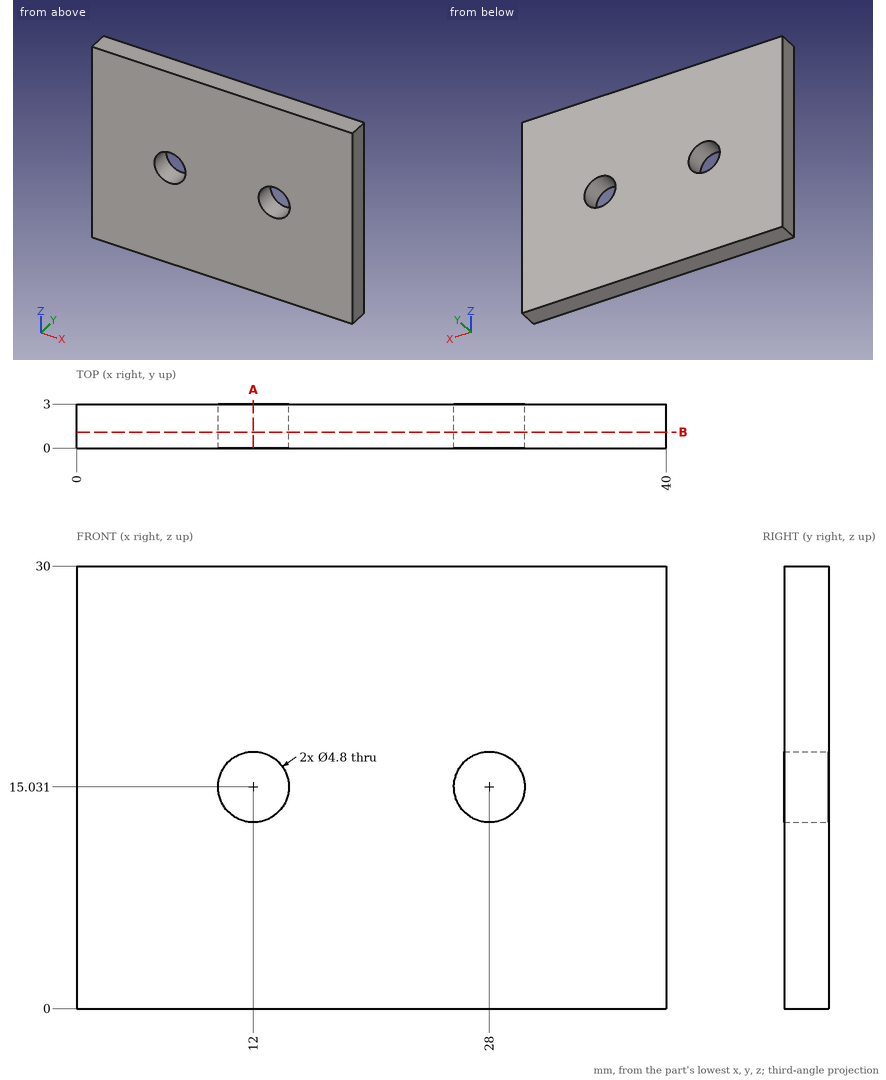
Geometry: see drawing. Coordinates: mm, zero at the bounding-box minimum. Coordinates: 2 decimals unless noted, no trailing zeros. Write each loop counter-clockwise with the first axis right and the second up, starting at its lowest first coordinate (ties: lowest second). Pieces come first, ordered by that corner, then holes. Notation, with made-up numbers: (26.25, 24.25) - (49.25, 24.25) arc R30 ccw to (49.25, 56.25) - close; hole circle Ø8 at (40, 67). An arc over 180 degrees is marked (long way). Put each result on its own line as item: value. Start each with the question number.
1) Ray query, L1, parallel to X at y = 1.65, z = 13.75; L2, parallel to Z at x = 27, y = 1.75; L3, parallel to Z at x = 29.5, y = 0.7. Return the intervals inside material, ascending.
2) Cut plane B-B (y = 1.1). Return the cut outline in (x, z), plus the area to 3 significant figures.
3) Cut plane A-A (x = 12). Return the cut outline in (y, z).
Resolved:
1. L1: x = 0 to 9.97, 14.03 to 25.97, 30.03 to 40
1. L2: z = 0 to 12.85, 17.21 to 30
1. L3: z = 0 to 13.16, 16.9 to 30
2. outline: (0, 0) - (40, 0) - (40, 30) - (0, 30) - close; hole circle Ø4.8 at (12, 15.03); hole circle Ø4.8 at (28, 15.03)
2. area: 1,160 mm2
3. outline: (0, 0) - (3, 0) - (3, 12.63) - (0, 12.63) - close; (0, 17.43) - (3, 17.43) - (3, 30) - (0, 30) - close
